Build history of the part. All positions in model axes, mm. Coordinates: 2 decimals unless noted, no trailing zeros. Order: outer loops, then holes, each group sorted by start corner. A loop starts at its lowest first (then second) coordinate and runs counter-clockwise, first axis right, second up. Notation, with made-up numbers: M -28,67 L 12,67 A27 ccw 12,83 Z; hole C 59.25,84 d5. An arc over 180 degrees is marked long. Write item = value, one per line. Start each with the question number.
Q1. Band-saw the part on B-B on x = -19.5. Write the cut outline in (y, z), plus the area to 3 significant figures.
Q2. Band-saw the part on D-D on z = 6.75. State how many separate pieces and enclosed holes the cut face has, plus the area to 3 significant figures.
Q3. Pin check, flat tips, straight feed: P1, Ø5, axis at x = -194.5, z = -2, coming from the +Y side; P2, Ø7.5, axis at x = 20.5, z = -1, coming from the +Y side; P3, Ø6, axis at x = -144.5, z = 5.5, coming from the -Y side. Stop position of each tip, or through.
Q4. Drill centre lines: probe 1 along Y at (x, z) = (7, -3.25); probe 2 along X at (y, z) = (0, 4); probe 3 along X at (y, z) = (11, 2). Where is each one in solid material? Low to high.
Q5. Band-saw the part on C-C on y = 0. Write the cut outline in (x, z).
Q6. Band-saw the part on A-A on y = 72.5. Write the cut outline in (x, z).
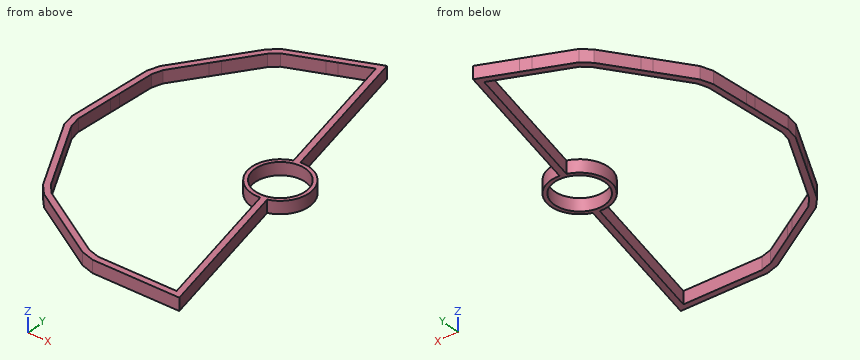
```python
from build123d import *

# Parameters (mm, degrees)
EXTRUDE_1_DEPTH     = 12.5
SKETCH_3_R          = 50
CUT_EXTRUDE_1_DEPTH = 40
SKETCH_4_R          = 57.5
SKETCH_4_R_2        = 50
EXTRUDE_2_DEPTH     = 25


with BuildPart() as part:
    # 草图1 → 凸台-拉伸1 (new, symmetric)
    with BuildSketch(Plane.XY):
        Polygon((10, -352), (85, -352), (-55.185850126, 349.743250156), (-124.732421354, 321.644611463), (-143.278173681, 314.151641145), (-212.824744909, 286.053002452), (-230.575847037, 270.460540253), (-275.085451102, 210.089181938), (-286.954678853, 193.990153053), (-331.464282918, 133.618794737), (-339.828804089, 110.704991943), (-346.104895164, 35.965016687), (-347.77851945, 16.034356619), (-354.054610525, -58.705618637), (-349.658052524, -83.739847979), (-315.841631523, -150.684982948), (-306.823919256, -168.53701894), (-273.007498256, -235.482153909), (-255.615985839, -255.285391269), (-191.736179852, -294.58451012), (-174.701564922, -305.064275147), (-110.821758935, -344.363393998), (-85, -352), (-10, -352), align=None)
        Polygon((-138.78289456, 303.02543489), (-206.438031879, 275.690985101), (-221.684684581, 262.298416336), (-265.426725534, 202.968155298), (-277.295953285, 186.869126414), (-320.782842839, 127.884944314), (-328.005353759, 108.099568976), (-334.146980853, 34.960882567), (-335.820605139, 15.030222499), (-341.966631122, -58.160848878), (-338.146174396, -79.914727665), (-305.130601702, -145.27445246), (-296.112889435, -163.126488451), (-262.984300248, -228.709947873), (-247.790635751, -246.010556193), (-185.448348981, -284.36378691), (-168.413734051, -294.843551937), (-105.890836047, -333.307895427), (-83.26273254, -340), (-10, -340), (10, -340), (70.365682758, -340), (-64.116651933, 333.192555096), (-120.237142233, 310.518405208), align=None, mode=Mode.SUBTRACT)
    extrude(amount=EXTRUDE_1_DEPTH, both=True)

    # 草图3 → 切除-拉伸1 (cut)
    with BuildSketch(Plane.XY.offset(12.5)):
        with Locations((8.563111146, 0)):
            Circle(SKETCH_3_R)
    extrude(amount=-CUT_EXTRUDE_1_DEPTH, mode=Mode.SUBTRACT)

    # 草图4 → 凸台-拉伸2 (add)
    with BuildSketch(Plane.XY.offset(12.5)):
        with Locations((8.563111146, 0)):
            Circle(SKETCH_4_R)
        with Locations((8.563111146, 0)):
            Circle(SKETCH_4_R_2, mode=Mode.SUBTRACT)
    extrude(amount=-EXTRUDE_2_DEPTH)


solid = part.part
```
Recorded:
q1.outline = M -352,-12.5 L -340,-12.5 L -340,12.5 L -352,12.5 Z; M -50.19,-12.5 L -41.38,-12.5 L -41.38,12.5 L -50.19,12.5 Z; M 41.38,-12.5 L 50.19,-12.5 L 50.19,12.5 L 41.38,12.5 Z; M 109.85,-12.5 L 171.11,-12.5 L 171.11,12.5 L 109.85,12.5 Z
q1.area = 2,270 mm2
q2.separate_pieces = 1
q2.enclosed_holes = 2
q2.area = 23,000 mm2
q3.P1 = 294.47
q3.P2 = 56.91
q3.P3 = -325.49
q4.probe_1 = -352 to -340, -57.48 to -49.98, 49.98 to 57.48
q4.probe_2 = -349.12 to -337.08, -48.94 to -41.44, 58.56 to 66.06
q4.probe_3 = -348.2 to -336.16, -47.87 to -40.21, 57.34 to 65
q5.outline = M -349.12,-12.5 L -337.08,-12.5 L -337.08,12.5 L -349.12,12.5 Z; M -48.94,-12.5 L -41.44,-12.5 L -41.44,12.5 L -48.94,12.5 Z; M 58.56,-12.5 L 66.06,-12.5 L 66.06,12.5 L 58.56,12.5 Z
q6.outline = M -343.04,-12.5 L -330.99,-12.5 L -330.99,12.5 L -343.04,12.5 Z; M -12.04,-12.5 L 0.2,-12.5 L 0.2,12.5 L -12.04,12.5 Z
